```python
from build123d import *

# Parameters (mm, degrees)
THREE_START                       = 19
THREE_ARMS_DEPTH                  = 19
CENTRE_BORE_SKETCH_R              = 10
CENTRE_BORE_DEPTH                 = 79
ARM_FILLETS_R10_A_R               = 10
ARM_FILLETS_R10_B_R               = 10
ARM_HOLE_1_SKETCH_R               = 3
ARM_HOLE_1_DEPTH                  = 79
ARM_HOLE_2_SKETCH_R               = 3
ARM_HOLE_2_DEPTH                  = 79
ARM_HOLE_3_SKETCH_R               = 3
ARM_HOLE_3_DEPTH                  = 79
ARM_CHAMFER_4MM_SIZE              = 4
BASE_C_BORE_HOLES_5_5_D           = 5.5
BASE_C_BORE_HOLES_5_5_DEPTH       = 9
BASE_C_BORE_HOLES_5_5_CBORE_D     = 9.5
BASE_C_BORE_HOLES_5_5_CBORE_DEPTH = 3


with BuildPart() as part:
    # Base Hub Profile → Base Hub (revolve)
    with BuildSketch(Plane.XY, mode=Mode.PRIVATE) as base_hub_sk:
        with BuildLine():
            Line((0, 0), (-20, 0))
            Line((-20, 0), (-20, 1))
            ThreePointArc((-20, 1), (-19.707106781, 1.707106781), (-19, 2))
            Line((-19, 2), (-17, 2))
            Line((-17, 2), (-17, 7))
            Line((-17, 7), (-31, 7))
            Line((-31, 7), (-31, 13))
            Line((-31, 13), (0, 13))
            Line((0, 13), (0, 0))
        make_face()
    revolve(base_hub_sk.sketch.rotate(Axis((0, 0, 0), (0, 1, 0)), 270), axis=Axis((0, 0, 0), (0, 1, 0)))

    # Arms Profile → Three Arms (add)
    with BuildSketch(Plane(origin=(0, 13, 0), x_dir=(1, 0, 0), z_dir=(0, 1, 0)).offset(THREE_START)):
        with BuildLine():
            Line((-5, 30.594117082), (-5, 2.886751274))
            Line((-5, 2.886751274), (-28.995282363, -10.966932145))
            ThreePointArc((-28.995282363, -10.966932145), (-29.806621866, -8.518526455), (-30.41161139, -6.011147367))
            Line((-30.41161139, -6.011147367), (-10, 5.773502549))
            Line((-10, 5.773502549), (-10, 29.342801502))
            ThreePointArc((-10, 29.342801502), (-7.526051267, 30.072554802), (-5, 30.594117082))
        make_face()
        with BuildLine():
            Line((5, 30.594117082), (5, 2.886751274))
            Line((5, 2.886751274), (28.995282363, -10.966932145))
            ThreePointArc((28.995282363, -10.966932145), (29.806621866, -8.518526455), (30.41161139, -6.011147367))
            Line((30.41161139, -6.011147367), (10, 5.773502549))
            Line((10, 5.773502549), (10, 29.342801502))
            ThreePointArc((10, 29.342801502), (7.526051267, 30.072554802), (5, 30.594117082))
        make_face()
        with BuildLine():
            Line((23.995282177, -19.627186076), (0, -5.773502764))
            Line((0, -5.773502764), (-23.995282177, -19.627186076))
            ThreePointArc((-23.995282177, -19.627186076), (-22.280570319, -21.554029467), (-20.411611017, -23.331655228))
            Line((-20.411611017, -23.331655228), (0, -11.547005527))
            Line((0, -11.547005527), (20.411611017, -23.331655228))
            ThreePointArc((20.411611017, -23.331655228), (22.280570319, -21.554029467), (23.995282177, -19.627186076))
        make_face()
    extrude(amount=-THREE_ARMS_DEPTH)

    # Centre Bore Sketch → Centre Bore (cut)
    with BuildSketch(Plane.XZ):
        with Locations(Location((0, 0, 0), (0, 0, 270))):
            Circle(CENTRE_BORE_SKETCH_R)
    extrude(amount=-CENTRE_BORE_DEPTH, mode=Mode.SUBTRACT)

    # Arm Fillets R10 A
    arm_fillets_r10_a_edges = [part.edges().sort_by_distance(p)[0] for p in [
        (-10, 22.5, -5.773502549),
    ]]
    fillet(arm_fillets_r10_a_edges, radius=ARM_FILLETS_R10_A_R)

    # Arm Fillets R10 B
    arm_fillets_r10_b_edges = [part.edges().sort_by_distance(p)[0] for p in [
        (0, 22.5, 11.547005527),
        (10, 22.5, -5.773502549),
    ]]
    fillet(arm_fillets_r10_b_edges, radius=ARM_FILLETS_R10_B_R)

    # Arm Hole 1 Sketch → Arm Hole 1 (cut)
    with BuildSketch(Plane(origin=(5.000000186, 0, 8.66025393), x_dir=(0.8660253930337038, 0, -0.5000000186208186), z_dir=(0.5000000186208186, 0, 0.8660253930337038))):
        with Locations((-21.342801502, 24)):
            Circle(ARM_HOLE_1_SKETCH_R)
    extrude(amount=-ARM_HOLE_1_DEPTH, mode=Mode.SUBTRACT)

    # Arm Hole 2 Sketch → Arm Hole 2 (cut)
    with BuildSketch(Plane.ZY.offset(10)):
        with Locations((-21.342801502, 24)):
            Circle(ARM_HOLE_2_SKETCH_R)
    extrude(amount=-ARM_HOLE_2_DEPTH, mode=Mode.SUBTRACT)

    # Arm Hole 3 Sketch → Arm Hole 3 (cut)
    with BuildSketch(Plane(origin=(5.000000186, 0, -8.66025393), x_dir=(-0.866025393033704, 0, -0.5000000186208184), z_dir=(0.5000000186208183, 0, -0.8660253930337038))):
        with Locations((-21.342801502, 24)):
            Circle(ARM_HOLE_3_SKETCH_R)
    extrude(amount=-ARM_HOLE_3_DEPTH, mode=Mode.SUBTRACT)

    # Arm Chamfer 4mm
    arm_chamfer_4mm_edges = [part.edges().sort_by_distance(p)[0] for p in [
        (-7.526051267, 32, -30.072554802),
        (-29.806621866, 32, 8.518526455),
        (-22.280570319, 32, 21.554029467),
        (22.280570319, 32, 21.554029467),
        (7.526051267, 32, -30.072554802),
        (29.806621866, 32, 8.518526455),
    ]]
    chamfer(arm_chamfer_4mm_edges, length=ARM_CHAMFER_4MM_SIZE)

    # Base C-Bore Holes Ø5.5
    with Locations(Plane(origin=(0, 13, 0), x_dir=(1, 0, 0), z_dir=(0, 1, 0))):
        with Locations((-17.67766953, 17.67766953), (0, -25), (17.67766953, 17.67766953)):
            CounterBoreHole(BASE_C_BORE_HOLES_5_5_D / 2, BASE_C_BORE_HOLES_5_5_CBORE_D / 2, BASE_C_BORE_HOLES_5_5_CBORE_DEPTH, depth=BASE_C_BORE_HOLES_5_5_DEPTH)


solid = part.part
```
Check sheet for the modelled part. Datum: model origin and axes. Units: mm. A direction names the side the tool comes from. Coordinates: 2 decimals unless noted, no trailing zeros. Loops run counter-clockwise (first coordinate to the right, second up) from the corner with the lowest first, then second, coordinate; pieces in that order, holes last.
1) Sectioned sample at B-B (y = 15). Record the boundary of the cut face in (x, z), and give its area (3 significant figures).
2) Access from +Z, -Z, +X, -X, +Y, -Y to the whole of each face (thin tool, end or side, straight path). Record for faces 1 (the face through (14.18, 11.52, -20.89)), 2 (the face through (-21, 13, -11)), 3 (the face through (-12.814, 20.522, 18.945)), 4 (the face through (-15.651, 8.479, -19.536)).
3) Material ranges on probe 1 along Y at (x, z) = (-13, -11.5); probe 2 along X at (y, z) = (23.5, 4); probe 3 along X at (y, z) = (21, -16.5), recorded low to high.
4) Gauge pin test, flat ends, axial feed: pin 1 (14 mm diameter, centred on y = 23.5, z = -17.5, fed in from -X); pin 2 (1.5 mm diameter, centred on y = 26.5, z = 12, fed in from -X); pin 3 (4.5 mm diameter, centred on x = 0, z = 25, fed in from +Y); pin 4 (8 mm diameter, centred on x = 21.5, z = 10, fed in from -Y). Record the tip position at first contact, or that the pin passes through.
5) Sectioned sample at A-A (x = 0). Record the boundary of the cut face in (y, z), and give its area (3 significant figures).
6) Sectioned sample at D-D (y = 4.5). Record the boundary of the cut face in (x, z).
7) Sectioned sample at C-C (z = 25). Record the boundary of the cut face in (x, y).
8) Release check for a two-part mould opening along X. For faces 5 (the face through (19.524, 0.507, 4.336)), 6 (the face through (-22.814, 20.522, 1.624)), 7 (the face through (-9, 0, -5)), 8 (the face through (0, 13, 20)) record: released by +X, released by -X, zero draft, split by the parting line, or undercut.
Check sheet entries:
1. outline: (-30.41, 6.01) - (-15, -2.89) arc R10 cw to (-10, -11.55) - (-10, -29.34) arc R31 ccw to (-5, -30.59) - (-5, -8.66) arc R10 cw to (-10, 0) - (-29, 10.97) arc R31 ccw to start; (-24, 19.63) - (-5, 8.66) arc R10 cw to (5, 8.66) - (24, 19.63) arc R31 ccw to (20.41, 23.33) - (5, 14.43) arc R10 cw to (-5, 14.43) - (-20.41, 23.33) arc R31 ccw to start; (5, -30.59) arc R31 ccw to (10, -29.34) - (10, -11.55) arc R10 cw to (15, -2.89) - (30.41, 6.01) arc R31 ccw to (29, 10.97) - (10, 0) arc R10 cw to (5, -8.66) - close
1. area: 717 mm2
2. face 1: +Y
2. face 2: -Z, -X, +Y
2. face 3: +Z, +Y
2. face 4: +Y, -Y
3. probe 1: y = 0 to 2, 7 to 13
3. probe 2: x = -26.93 to -25.75, -18.92 to -16.93, 16.93 to 18.92, 25.75 to 26.93
3. probe 3: x = -10 to -5, 5 to 10
4. pin 1: stops at x = -10.05
4. pin 2: stops at x = -12.08
4. pin 3: passes through
4. pin 4: stops at y = 0
5. outline: (0, -20) - (1, -20) arc R1 ccw to (2, -19) - (2, -17) - (7, -17) - (7, -31) - (13, -31) - (13, -10) - (0, -10) - close; (0, 10) - (32, 10) - (32, 13.09) - (13, 13.09) - (13, 20.25) - (10, 20.25) - (10, 22.25) - (7, 22.25) - (7, 17) - (2, 17) - (2, 19) arc R1 ccw to (1, 20) - (0, 20) - close; (7, 27.75) - (10, 27.75) - (10, 29.75) - (13, 29.75) - (13, 31) - (7, 31) - close
5. area: 375 mm2
6. outline: circle Ø34 at (0, 0); hole circle Ø20 at (0, 0)
7. outline: (-18.33, 7) - (-2.75, 7) - (-2.75, 10) - (-4.75, 10) - (-4.75, 13) - (-18.33, 13) - close; (2.75, 7) - (18.33, 7) - (18.33, 13) - (4.75, 13) - (4.75, 10) - (2.75, 10) - close
8. face 5: split by the parting line
8. face 6: released by -X
8. face 7: zero draft
8. face 8: undercut
